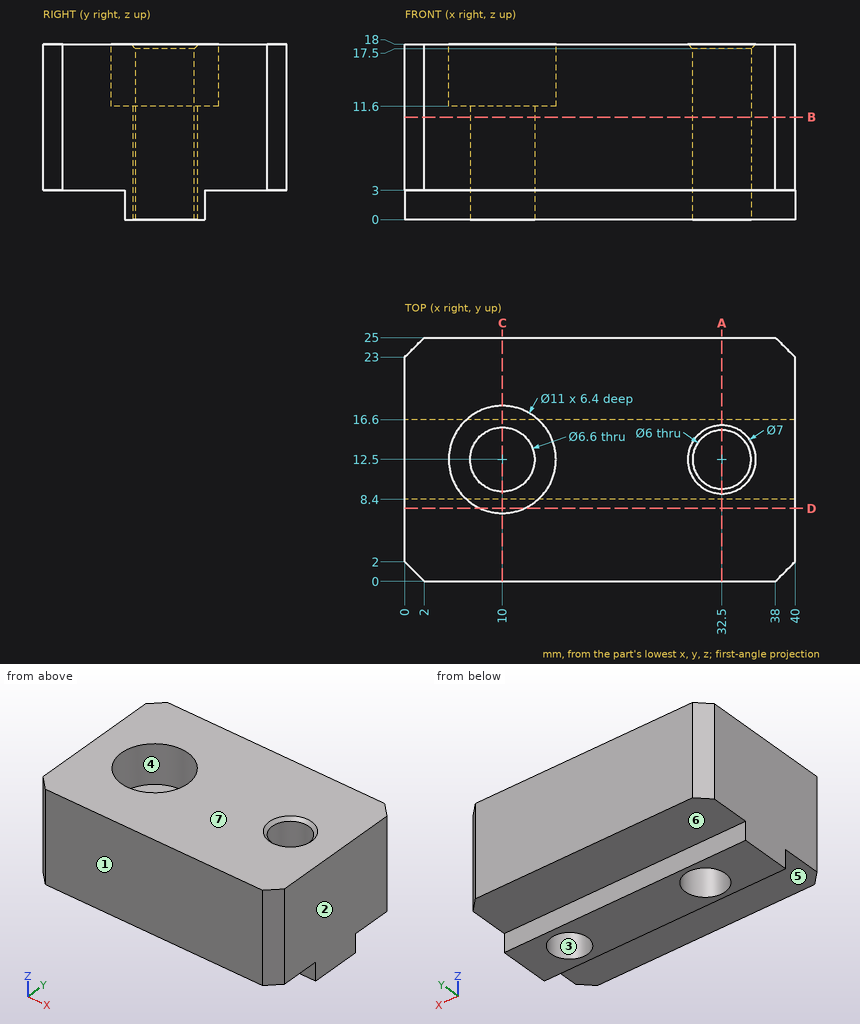
Can you work these out from the drawing? Everything is in mm from the part's minimum corner. A direction names the side the tool comes from. Give positions to 0.01 mm unless a question says otherwise; leave off trailing zeros. Loops run counter-clockwise (first coordinate to the right, second up) from the corner with the lowest first, then second, coordinate; pieces in that order, holes last. Notation, with made-up numbers: M 79.5,20 L 129.5,20 A16 cw 129.5,34 Z; hole C 42.25,-26 d2. An arc over 180 degrees is marked long. Put each result on its own line as item: value. Start each with the question number.
(1) I want a section at A-A on x = 32.5. Please give me the cut outline in (y, z).
(2) If we mould it in two halves opening along Y, with no side actions, what happens to the marked faces 1, 2, 3 and 4? For each: +Y half, -Y half, draft (parallel to the pull), parting line (faces both ways), or undercut.
(3) Will these pins go through, and if not, where does the flat tip stop? pin 1 Ø4 at (x, y) = (15.5, 20) entering from -Z; pin 2 Ø3.5 at (x, y) = (11.5, 11.5) entering from +Z; pin 3 Ø3.5 at (x, z) = (16, 1) entering from -Y; pin 4 Ø6.5 at (x, y) = (10, 12.5) entering from -Z.
(4) I want a section at D-D on y = 7.5. Please give me the cut outline in (x, z).
(5) I want a section at C-C on x = 10. Please give me the cut outline in (y, z).
(6) I need wall thicknesses on line 1 along Y through (x, z) = (10, 6); line 2 along Y through (x, z) = (10, 13.25); line 3 along Y through (x, z) = (25.5, 1.75). Which ranges of each line are inside material? Lowest first, please. Write a range as [from, to].
(7) For the marked faces 5, 6 and 7, which set-ups out of +Z, -Z, +X, -X, +Y, -Y let a thin tool reach every point of the face, with its end or its side?
(8) I want a section at B-B on z = 10.5. Please give me the cut outline in (x, y).
Answer block:
1. outline: M 0,3 L 8.4,3 L 8.4,0 L 9.5,0 L 9.5,17.5 L 9,18 L 0,18 Z; M 15.5,0 L 16.6,0 L 16.6,3 L 25,3 L 25,18 L 16,18 L 15.5,17.5 Z
2. face 1: -Y half
2. face 2: draft
2. face 3: undercut
2. face 4: undercut
3. pin 1: z = 3
3. pin 2: z = 11.6
3. pin 3: y = 8.4
3. pin 4: through
4. outline: M 0,3 L 40,3 L 40,18 L 12.29,18 L 12.29,11.6 L 7.71,11.6 L 7.71,18 L 0,18 Z
5. outline: M 0,3 L 8.4,3 L 8.4,0 L 9.2,0 L 9.2,11.6 L 7,11.6 L 7,18 L 0,18 Z; M 15.8,0 L 16.6,0 L 16.6,3 L 25,3 L 25,18 L 18,18 L 18,11.6 L 15.8,11.6 Z
6. line 1: [0, 9.2], [15.8, 25]
6. line 2: [0, 7], [18, 25]
6. line 3: [8.4, 16.6]
7. face 5: -Z, +X, -X, -Y
7. face 6: -Z, +X, -X, +Y
7. face 7: +Z, +X, -X, +Y, -Y
8. outline: M 0,2 L 2,0 L 38,0 L 40,2 L 40,23 L 38,25 L 2,25 L 0,23 Z; hole C 10,12.5 d6.6; hole C 32.5,12.5 d6
